from build123d import *

# Parameters (mm, degrees)
SKETCH_1_W         = 40
SKETCH_1_H         = 40
EXTRUDE_1_DEPTH    = 4
FILLET_1_R         = 10
HOLE_WIZARD_M6_1_D = 6.6


with BuildPart() as part:
    # 草图1 → 凸台-拉伸1 (new body)
    with BuildSketch(Plane.XY):
        Rectangle(SKETCH_1_W, SKETCH_1_H)
    extrude(amount=EXTRUDE_1_DEPTH)

    # 圆角1
    fillet_1_edges = [part.edges().sort_by_distance(p)[0] for p in [
        (20, -20, 2),
        (-20, -20, 2),
        (-20, 20, 2),
        (20, 20, 2),
    ]]
    fillet(fillet_1_edges, radius=FILLET_1_R)

    # Hole Wizard M6 _1 (through all)
    with Locations(Plane(origin=(0, 0, 0), x_dir=(-1, 0, 0), z_dir=(0, 0, -1))):
        with Locations((0, 0)):
            Hole(HOLE_WIZARD_M6_1_D / 2)


solid = part.part
Build history of the part. All positions in model axes, mm. Give positions to 0.01 mm unless a question says otherwise; leave off trailing zeros. Order: outer loops, then holes, each group sorted by start corner. A loop starts at its lowest first (then second) coordinate and runs counter-clockwise, first axis right, second up. Notation, with made-up numbers: M 32.25,-29 L 38.25,-29 A18 cw 38.25,-18 Z; hole C 59,-22 d5. An arc over 180 degrees is marked long. Put each result on its own line as item: value.
Item 1: Cut at A-A on y = 0. Write the cut outline in (x, z).
Results are:
outline: M -20,0 L -3.3,0 L -3.3,4 L -20,4 Z; M 3.3,0 L 20,0 L 20,4 L 3.3,4 Z
Item 2: Cut at D-D on x = 17.5. Write the cut outline in (y, z), then the cut area to 3 significant figures.
Results are:
outline: M -16.61,0 L 16.61,0 L 16.61,4 L -16.61,4 Z
area: 133 mm2
Item 3: Wall check: probe 1 along Y at (x, z) = (0, 2.85); probe 2 along X at (y, z) = (3, 1.1); probe 3 along X at (y, z) = (15, 1.2). Give the ranges that are in metal, low to high.
Results are:
probe 1: -20 to -3.3, 3.3 to 20
probe 2: -20 to -1.37, 1.37 to 20
probe 3: -18.66 to 18.66
Item 4: Cut at C-C on z = 3.3. Write the cut outline in (x, y).
Results are:
outline: M -20,-10 A10 ccw -10,-20 L 10,-20 A10 ccw 20,-10 L 20,10 A10 ccw 10,20 L -10,20 A10 ccw -20,10 Z; hole C 0,0 d6.6
Item 5: Pull direction Y, two halves, no side cores. Call faces 1 (the face through (-2.43, 2.23, 2.03)), 2 (the face through (0, 20, 2)), 3 (the face through (-20, 0, 2)): +Y half, -Y half, draft (parallel to the pull), parting line (faces both ways), or undercut.
Results are:
face 1: undercut
face 2: +Y half
face 3: draft
Item 6: Drop a flat-ended pin along its axis: pin 1 Ø2 at (x, z) = (-13, 2) entering from -Y. Give the stop position or say it passes through.
Results are:
pin 1: y = -19.8
